Could you check a few things on this model? Use its own coordinates, in mm. A direction names the side the tool comes from. Coordinates: 2 decimals unless noted, no trailing zeros. Order: outer loops, then holes, each group sorted by start corner. A loop starts at its lowest first (then second) coordinate and runs counter-clockwise, first axis right, second up. Notation, with made-up numbers: M 75.25,-14.75 L 83.25,-14.75 A16 cw 83.25,-7.75 Z; hole C 60.5,-17.5 d6. An arc over 180 degrees is marked long. One line per question, with ' | ' between items. Start each with the question number.
from build123d import *

# Parameters (mm, degrees)
BOSS_EXTRUDE1_DEPTH = 342.5
SKETCH2_W           = 15
SKETCH2_H           = 75
BOSS_EXTRUDE2_DEPTH = 57.5
SKETCH3_R           = 13
CUT_EXTRUDE1_DEPTH  = 57.5


with BuildPart() as part:
    # Sketch1 → Boss-Extrude1 (new, symmetric)
    with BuildSketch(Plane(origin=(0, 0, 0), x_dir=(1, 0, 0), z_dir=(0, 1, 0))):
        Polygon((0, -37.5), (0, 37.5), (10, 42.881796684), (65, 60), (65, 45), (30, 35), (30, -35), (65, -45), (65, -60), (10, -42.881796684), align=None)
    extrude(amount=BOSS_EXTRUDE1_DEPTH, both=True)

    # Sketch2 → Boss-Extrude2 (add)
    with BuildSketch(Plane.XZ.offset(342.5)):
        with Locations((7.5, 0)):
            Rectangle(SKETCH2_W, SKETCH2_H)
    boss_extrude2 = extrude(amount=BOSS_EXTRUDE2_DEPTH)

    # Mirror1: Boss-Extrude2 across plane
    add(boss_extrude2.mirror(Plane.ZX))

    # Sketch3 → Cut-Extrude1 (cut)
    with BuildSketch(Plane.ZY):
        with Locations((0, 377.5)):
            Circle(SKETCH3_R)
        with Locations((0, -377.5)):
            Circle(SKETCH3_R)
    extrude(amount=-CUT_EXTRUDE1_DEPTH, mode=Mode.SUBTRACT)


solid = part.part
(1) Imagine slicing it at B-B, the plane z = 0. Write out the boundary of the cut face in (x, y).
(2) Imagine slicing it at C-C, the plane x = 52. Write out the boundary of the cut face in (y, z).
(3) Imagine slicing it at A-A, the plane y = -377.5. Write out the boundary of the cut face in (x, z).
(4) We'd pull the mould along Y, two halves only. Please class faces 1 (the flat face through (7, -400, 1)), 2 (the flat face through (7, 400, 1)), 3 (the flat face through (0, -6, -1)), 4 (the cylindrical face through (7.4, -390.19, -2.82)): +Y half, -Y half, draft (parallel to the pull), parting line (faces both ways), or undercut.
(5) Imagine slicing it at D-D, the plane y = -277. Write out the boundary of the cut face in (x, z).
(6) If I drill on line 1 along Y through (x, z) = (6.5, 0); line 2 along Y through (x, z) = (12.5, -10.5); line 3 along Z through (x, y) = (5, -377), over which ranges is the centre line in solid material (lowest first)? Write a range as from..to.
(7) For P1, Ø15.5, axis at y = -377.5, z = 0, coming from the -X side; P2, Ø2, axis at x = 48.5, y = 118.5, coming from the -Z side; P3, Ø16.5, axis at x = 6, y = -378.5, coming from the +Z side; P4, Ø6, axis at x = 45.5, y = 207, coming from the -Z side, each with a flat end and sliding along its axis, tell me the tip position at first contact or that it passes through.
(8) On a 3-axis mill with a long thin cutter (end or side, diameter ignored), from which of +Z, -Z, +X, -X, +Y, -Y can I reach the whole of each face in a straight line? I mean faces 5 (the flat face through (47.74, 4.8, -40.07)), 6 (the flat face through (15, -364, -1)), 7 (the flat face through (7, -371, 37.5)). Say none if no direction works.
Answers:
1) outline: M 0,-400 L 15,-400 L 15,-390.5 L 0,-390.5 Z; M 0,-364.5 L 15,-364.5 L 15,-342.5 L 30,-342.5 L 30,342.5 L 15,342.5 L 15,364.5 L 0,364.5 Z; M 0,390.5 L 15,390.5 L 15,400 L 0,400 Z
2) outline: M -342.5,-55.95 L 342.5,-55.95 L 342.5,-41.29 L -342.5,-41.29 Z; M -342.5,41.29 L 342.5,41.29 L 342.5,55.95 L -342.5,55.95 Z
3) outline: M 0,-37.5 L 15,-37.5 L 15,-13 L 0,-13 Z; M 0,13 L 15,13 L 15,37.5 L 0,37.5 Z
4) face 1: -Y half | face 2: +Y half | face 3: draft | face 4: undercut
5) outline: M 0,-37.5 L 10,-42.88 L 65,-60 L 65,-45 L 30,-35 L 30,35 L 65,45 L 65,60 L 10,42.88 L 0,37.5 Z
6) line 1: -400..-390.5, -364.5..364.5, 390.5..400 | line 2: -400..-385.16, -369.84..369.84, 385.16..400 | line 3: -37.5..-12.99, 12.99..37.5
7) P1: through | P2: z = -55.18 | P3: z = 37.5 | P4: z = -54.86
8) face 5: +X, +Y, -Y | face 6: +Z, -Z, +X, -Y | face 7: +Z, +X, -X, -Y
